The drawing under review shows one solid part. Ordinate dimensions are in mm from its lowest x, y, z. A direction names the side the tool comes from. Round coordinates to 2 decimals unless told otherwise and drop trailing zeros. Order: outer loops, then holes, each group sorted by start corner. A loop starts at its lowest first (then second) coordinate and runs counter-clockwise, first axis right, second up.
1) Clearance check with flat-ended pins moving along their axes: P1, Ø1.5, axis at y = 46.5, z = 4.5, coming from the +X side; P2, Ø5.5, axis at x = 75, z = 7.5, coming from the +Y side; P3, Ø4, axis at y = 54, z = 9.5, coming from the -X side. State where each tip first meets the part, or that it passes through.
2) To check wall thickness, follow L1, parallel to X at y = 64.75, z = 7.5; L2, parallel to Y at x = 60, z = 6; L3, parallel to Y at x = 74.5, z = 1.25 (3 decimals). State the ranges of each line that lie inside material, in increasing order.
3) Consider section B-B (x = 20). Give the boundary of the cut face in (y, z).
4) Consider section A-A (z = 9.75). Give the number of separate pieces and of enclosed holes in the cut face, then the cut area to 3 significant figures.
5) Consider section C-C (y = 20). Give the boundary of the cut face in (x, z).
6) Mouldability with a two-part tool opening along Y and no side actions: class the marked faces 6, 7, 8 and 9 as pulls with the +Y half, pulls with the -Y half, needs draft (parallel to the pull), parting line crosses it, or undercut.
7) Machinability: for the marked faces 1, 2, 3, 4 and 5, which of the approach directions +Z, -Z, +X, -X, +Y, -Y give a long, thin tool a straight path to every point of the face, cutting with its end or side? Answer none if there is none.
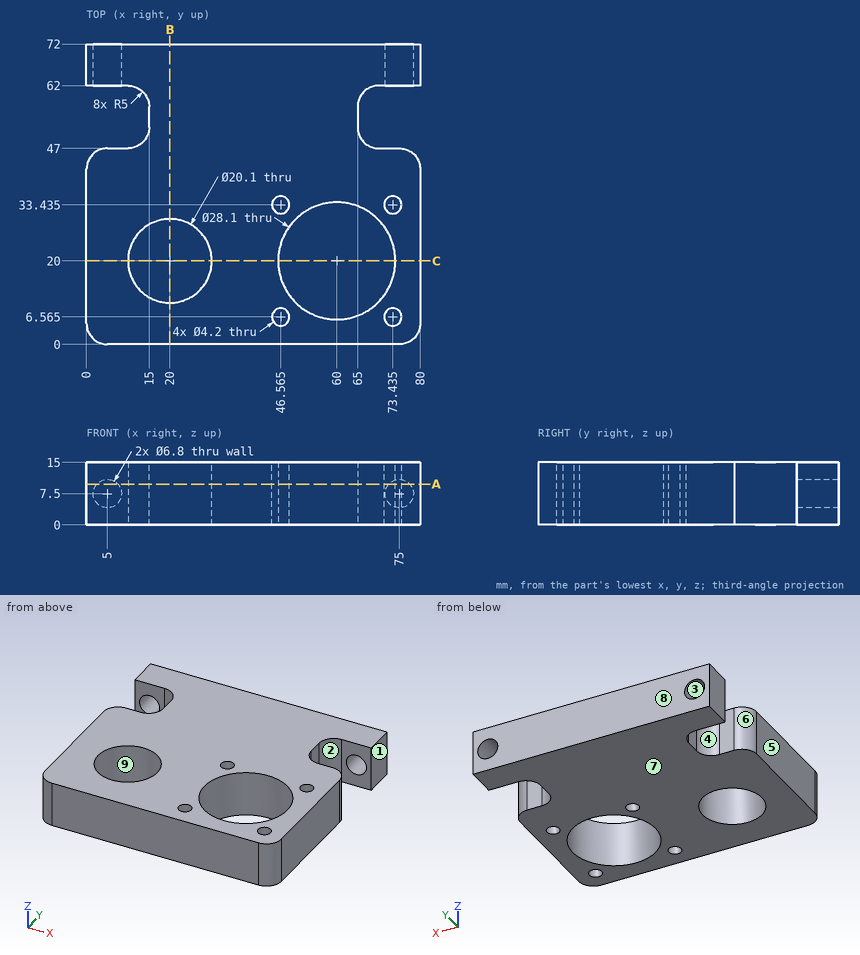
Answer below:
1. P1: stops at x = 78.31
1. P2: stops at y = 47
1. P3: stops at x = 15
2. L1: x = 0 to 1.6, 8.4 to 71.6, 78.4 to 80
2. L2: y = 0 to 5.95, 34.05 to 72
2. L3: y = 0 to 4.755, 8.375 to 31.625, 35.245 to 47, 62 to 72
3. outline: (0, 0) - (9.95, 0) - (9.95, 15) - (0, 15) - close; (30.05, 0) - (72, 0) - (72, 15) - (30.05, 15) - close
4. separate pieces: 3
4. enclosed holes: 6
4. area: 4,220 mm2
5. outline: (0, 0) - (9.95, 0) - (9.95, 15) - (0, 15) - close; (30.05, 0) - (45.95, 0) - (45.95, 15) - (30.05, 15) - close; (74.05, 0) - (80, 0) - (80, 15) - (74.05, 15) - close
6. face 6: undercut
6. face 7: needs draft
6. face 8: pulls with the +Y half
6. face 9: undercut
7. face 1: +Z, -Z, +X, +Y, -Y
7. face 2: +Z, -Z, +X
7. face 3: +Y
7. face 4: +Z, -Z, -X
7. face 5: +Z, -Z, -X, +Y, -Y
